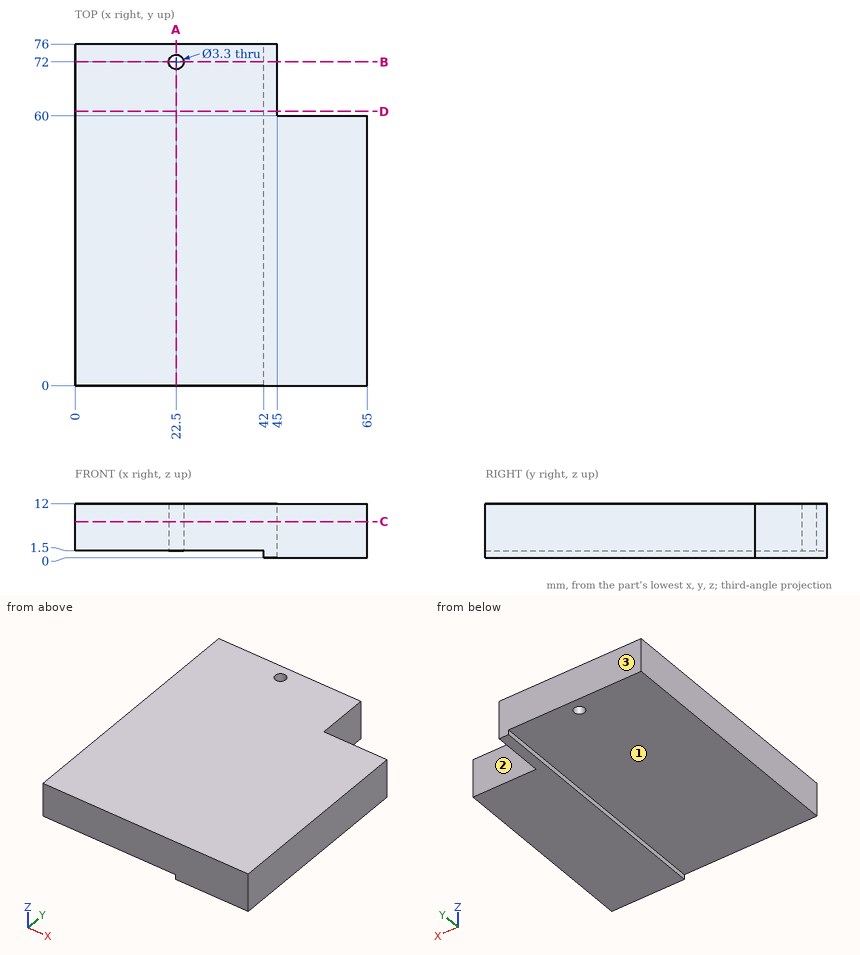
Input: dimensioned drawing with shaded views. Units: mm. Origin: part minimum x, y, z. A direction names the side the tool comes from. Give positions to 0.01 mm unless a question says otherwise; leave off trailing zeros. Write each loop counter-clockwise with the first axis right and the second up, starting at its lowest first coordinate (ties: lowest second). Pieces come first, ordered by that corner, then holes.
1. Section query D-D (y = 61). Return the cut outline in (x, z), then the cut area to 3 significant figures.
2. Material intervals for line 1 along Y through (x, z) = (22.5, 9); line 2 along X through (y, z) = (72, 5.25); line 3 along Z through (x, y) = (40, 6), sorted ascending.
3. First-contact query: pin 1 (8 mm diameter, centred on x = 39.5, y = 53, fed in from -Z); pin 2 (2.5 mm diameter, centred on x = 22.5, y = 72, fed in from -Z) (3 decimals); pin 3 (0.8 mm diameter, centred on y = 19, z = 1, fed in from -X); pin 4 (21 mm diameter, centred on x = 23.5, y = 57, fed in from -Z). Flat tips, straight axial feed; report the tip coordinate or a pass-through.
4. Section query A-A (x = 22.5). Return the cut outline in (y, z), then the cut area to 3 significant figures.
5. Section query B-B (y = 72). Return the cut outline in (x, z).
6. Access query for the marked faces 1, 2 and 3. Directions: +Z, -Z, +X, -X, +Y, -Y. A direction counts if a zero-diameter tool reaches every point of the face in a straight line with its end or side. Return the directions, or none.
7. Section query C-C (z = 8). Return the cut outline in (x, y), then the cut area to 3 significant figures.
Output values:
1. outline: (0, 1.5) - (42, 1.5) - (42, 0) - (45, 0) - (45, 12) - (0, 12) - close
1. area: 477 mm2
2. line 1: y = 0 to 70.35, 73.65 to 76
2. line 2: x = 0 to 20.85, 24.15 to 45
2. line 3: z = 1.5 to 12
3. pin 1: stops at z = 0
3. pin 2: passes through
3. pin 3: stops at x = 42
3. pin 4: stops at z = 1.5
4. outline: (0, 1.5) - (70.35, 1.5) - (70.35, 12) - (0, 12) - close; (73.65, 1.5) - (76, 1.5) - (76, 12) - (73.65, 12) - close
4. area: 763 mm2
5. outline: (0, 1.5) - (20.85, 1.5) - (20.85, 12) - (0, 12) - close; (24.15, 1.5) - (42, 1.5) - (42, 0) - (45, 0) - (45, 12) - (24.15, 12) - close
6. face 1: -Z, -X, +Y, -Y
6. face 2: +Z, -Z, +X, +Y
6. face 3: +Z, -Z, +X, -X, +Y
7. outline: (0, 0) - (65, 0) - (65, 60) - (45, 60) - (45, 76) - (0, 76) - close; hole circle Ø3.3 at (22.5, 72)
7. area: 4,610 mm2
